```python
from build123d import *


with BuildPart() as part:
    # Sketch1 → Revolve1 (revolve)
    with BuildSketch(Plane(origin=(0, 0, 0), x_dir=(1, 0, 0), z_dir=(0, 1, 0))):
        Polygon((4.7, 0), (5.53, 0), (5.73, 0.2), (5.73, 9.8), (5.53, 10), (4.7, 10), (4.5, 9.8), (4.5, 6), (3.5, 6), (3.5, 4), (4.5, 4), (4.5, 0.2), align=None)
    revolve(axis=Axis((0, 0, 0), (0, 0, -1)))


solid = part.part
```
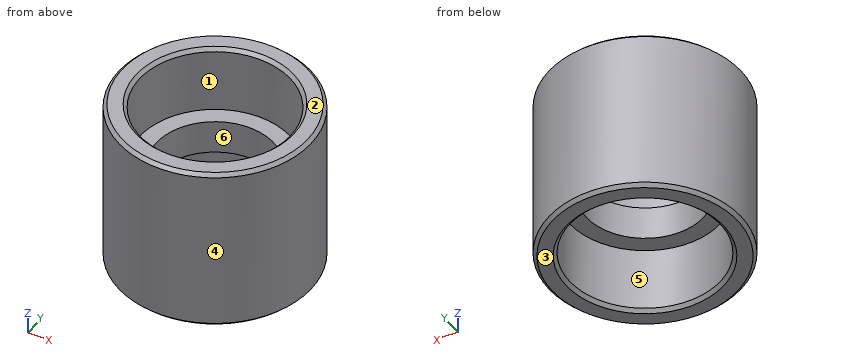
Check sheet for the modelled part. Datum: model origin and axes. Units: mm. Face numbers are marked on the shaded views. A direction names the side the tool comes from. Round coordinates to 2 decimals unless told otherwise and drop trailing zeros. Loops run counter-clockwise (first coordinate to the right, second up) from the corner with the lowest first, then second, coordinate; pieces in that order, holes last. Notation, with made-up numbers: (6, 72) - (47, 72) arc R28 cw to (47, 95) - close; hole circle Ø7 at (-3.75, -14.5). An arc over 180 degrees is marked (long way). Answer as a JSON object with one key per item and string values. Group by question number.
Q1. Sectioned sample at D-D, the plane z = -1.5. Enter the section's corners in (x, y).
Q2. Set-up check for the marked faces 1 and 2: record each of +Z, -Z, +X, -X, +Y, -Y from which the full face is reachable in a straight line by a thin tool's end or side.
Q3. Mould release check, pull along X, two halves, no side actions. Record for the marked faces 3, 4, 5 and 6: released by +X, released by -X, zero draft, split by the parting line, or undercut.
Q4. Sectioned sample at A-A, the plane x = 0. Enter the section's corners in (y, z), plus the area to 3 significant figures.
Q5. Gauge pin test, flat ends, axial feed: P1, Ø4.5, axis at x = -1, y = -1, coming from the +Z side; P2, Ø1.5, axis at y = 1.5, z = -8, coming from the -X side; P3, Ø5.5, axis at x = 0, y = 0, coming from the -Z side; P4, Ø5, axis at x = 4, z = -7, coming from the -Y side. Record the tip position at first contact, or that the pin passes through.
Q6. Scan lines: line 1 along Y through (x, z) = (0, -8.4); line 2 along X through (y, z) = (0, -4.65). Record each from-to range of solid material in increasing order. Write a range as [from, to].
Q7. Sectioned sample at C-C, the plane z = -4.25. Enter the section's corners in (x, y), plus the area to 3 significant figures.
Solution:
{
 "1": {"outline": "circle Ø11.46 at (0, 0); hole circle Ø9 at (0, 0)"},
 "2": {"face 1": "+Z", "face 2": "+Z, +X, -X, +Y, -Y"},
 "3": {"face 3": "zero draft", "face 4": "split by the parting line", "face 5": "undercut", "face 6": "undercut"},
 "4": {"outline": "(-5.73, -9.8) - (-5.53, -10) - (-4.7, -10) - (-4.5, -9.8) - (-4.5, -6) - (-3.5, -6) - (-3.5, -4) - (-4.5, -4) - (-4.5, -0.2) - (-4.7, 0) - (-5.53, 0) - (-5.73, -0.2) - close; (3.5, -6) - (4.5, -6) - (4.5, -9.8) - (4.7, -10) - (5.53, -10) - (5.73, -9.8) - (5.73, -0.2) - (5.53, 0) - (4.7, 0) - (4.5, -0.2) - (4.5, -4) - (3.5, -4) - close", "area": "28.4 mm²"},
 "5": {"P1": "stops at z = -4", "P2": "stops at x = -5.68", "P3": "passes through", "P4": "stops at y = -5.53"},
 "6": {"line 1": "y = [-5.73, -4.5], [4.5, 5.73]", "line 2": "x = [-5.73, -3.5], [3.5, 5.73]"},
 "7": {"outline": "circle Ø11.46 at (0, 0); hole circle Ø7 at (0, 0)", "area": "64.7 mm²"}
}
